Check sheet for the drawn part. Datum: minimum x, y, z corner. Units: mm. Round coordinates to 2 decimals unless told otherwise and drop trailing zeros. Order: outer loops, then holes, each group sorted by start corner. A loop starts at its lowest first (then second) coordinate and runs counter-clockwise, first axis right, second up. Notation, with made-up numbers: (-19, 15) -> (11, 15) arc R19 ccw to (11, 20) -> close; hole circle Ø11 at (18.5, 42). An arc over 180 degrees is marked (long way). Answer in a Markdown table with one row per item.
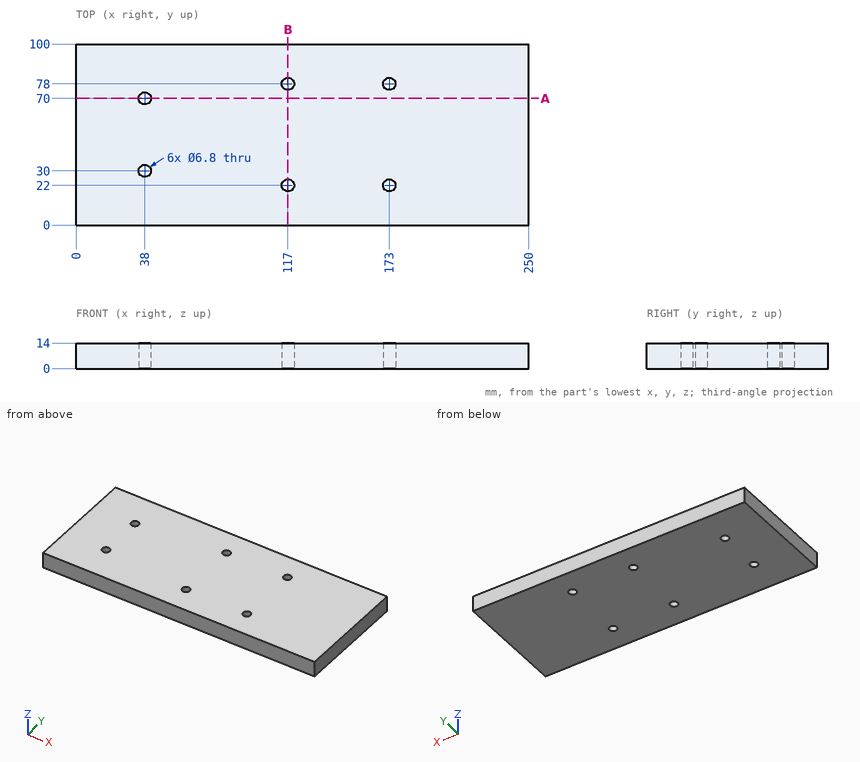
(1) Depth check by flat-ended pin: pin 1 Ø6 at (x, y) = (173, 78) entering from -Z (3 decimals). Enter the tip coordinate at first touch or a pass-through.
Solutions:
| item | result |
|---|---|
| pin 1 | through |
(2) Scan lines: probe 1 along Y at (x, z) = (38, 9); probe 2 along Y at (x, z) = (115, 7.25); probe 3 along X at (y, z) = (23.5, 1.75). Record each from-to range of solid material in increasing order. Write a range as from..to.
Solutions:
| item | result |
|---|---|
| probe 1 | 0..26.6, 33.4..66.6, 73.4..100 |
| probe 2 | 0..19.25, 24.75..75.25, 80.75..100 |
| probe 3 | 0..113.95, 120.05..169.95, 176.05..250 |
(3) Section check A-A on y = 70. Record the boundary of the cut face in (x, z).
Solutions:
| item | result |
|---|---|
| outline | (0, 0) -> (34.6, 0) -> (34.6, 14) -> (0, 14) -> close; (41.4, 0) -> (250, 0) -> (250, 14) -> (41.4, 14) -> close |
(4) Section check B-B on x = 117. Record the boundary of the cut face in (y, z).
Solutions:
| item | result |
|---|---|
| outline | (0, 0) -> (18.6, 0) -> (18.6, 14) -> (0, 14) -> close; (25.4, 0) -> (74.6, 0) -> (74.6, 14) -> (25.4, 14) -> close; (81.4, 0) -> (100, 0) -> (100, 14) -> (81.4, 14) -> close |
